Source: CAD feature listing. Evaluate the final solid. Frame: model axes, mm. Face numbers are marked on the shaded views. Give positions to 0.01 mm unless a question says otherwise; leave off trailing zeros. Loops run counter-clockwise (first coordinate to the right, second up) from the corner with the lowest first, then second, coordinate; pieces in that order, holes last. Notation, with made-up numbers: (9.25, 64) -> (33.25, 64) arc R5 ccw to (33.25, 68) -> close; hole circle Ø2 at (71, 17.25). An arc over 180 degrees is marked (long way). Put each result on its own line as item: value.
```python
from build123d import *

# Parameters (mm, degrees)
CHAMFER1_SIZE = 1


with BuildPart() as part:
    # Sketch1 → Revolve2 (revolve)
    with BuildSketch(Plane.XY, mode=Mode.PRIVATE) as revolve2_sk:
        with BuildLine():
            Line((-2, 0), (-2, 25.291796068))
            ThreePointArc((-2, 25.291796068), (-5.61248608, 27.816699867), (-7, 32))
            Line((-7, 32), (-8, 32))
            Line((-8, 32), (-8, 10))
            Line((-8, 10), (-4, 10))
            Line((-4, 10), (-4, 0))
            Line((-4, 0), (-2, 0))
        make_face()
    revolve(revolve2_sk.sketch.rotate(Axis((0, 0, 0), (0, 1, 0)), 270), axis=Axis((0, 0, 0), (0, 1, 0)))

    # Chamfer1
    chamfer1_edges = [part.edges().sort_by_distance(p)[0] for p in [
        (0, 10, 8),
        (0, 0, 4),
    ]]
    chamfer(chamfer1_edges, length=CHAMFER1_SIZE)


solid = part.part
```
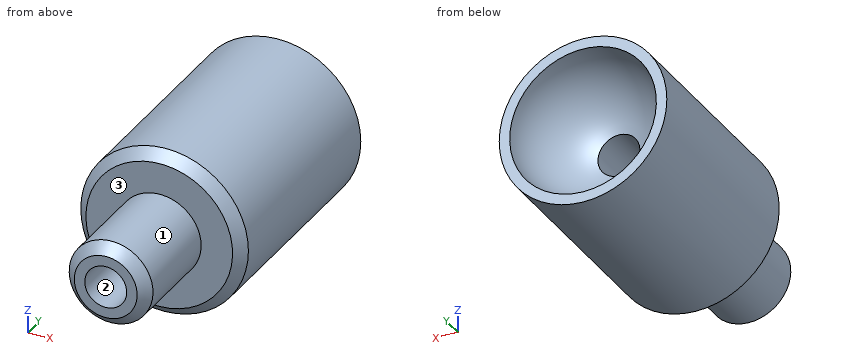
(1) Section B-B on z = 0. Return loops of the section in (x, y), then the cut area to 3 significant figures.
Calculated:
outline: (-8, 11) -> (-7, 10) -> (-4, 10) -> (-4, 1) -> (-3, 0) -> (-2, 0) -> (-2, 25.29) arc R7 cw to (-7, 32) -> (-8, 32) -> close; (2, 0) -> (3, 0) -> (4, 1) -> (4, 10) -> (7, 10) -> (8, 11) -> (8, 32) -> (7, 32) arc R7 cw to (2, 25.29) -> close
area: 253 mm²
(2) Draft query along Z for the marked faces 1, 2 and 3. Return one class per face: released by +Z, released by -Z, zero draft, split by the parting line, or undercut.
Calculated:
face 1: split by the parting line
face 2: undercut
face 3: zero draft
(3) First-contact query: P1, Ø6, axis at x = -1.5, y = 6, coming from the -Z side. Flat tip, straight axial feed; report the tip coordinate or a pass-through.
Calculated:
P1: stops at z = -4
(4) Section C-C on y = 6. Return loops of the section in (x, z), then the cut area to 3 significant figures.
Calculated:
outline: circle Ø8 at (0, 0); hole circle Ø4 at (0, 0)
area: 37.7 mm²
(5) Section D-D on y = 21. Return loops of the section in (x, z).
Calculated:
outline: circle Ø16 at (0, 0); hole circle Ø4 at (0, 0)
(6) Line query: probe 1 along X at (y, z) = (18.75, 0); probe 2 along X at (y, z) = (7.75, 0); probe 3 along Z at (x, y) = (1.25, 5.5). Output: solid intervals per line, ascending. Write a range as from..to.
Calculated:
probe 1: x = -8..-2, 2..8
probe 2: x = -4..-2, 2..4
probe 3: z = -3.8..-1.56, 1.56..3.8
(7) Section A-A on x = 0. Return loops of the section in (y, z).
Calculated:
outline: (0, -3) -> (1, -4) -> (10, -4) -> (10, -7) -> (11, -8) -> (32, -8) -> (32, -7) arc R7 cw to (25.29, -2) -> (0, -2) -> close; (0, 2) -> (25.29, 2) arc R7 cw to (32, 7) -> (32, 8) -> (11, 8) -> (10, 7) -> (10, 4) -> (1, 4) -> (0, 3) -> close
